```python
from build123d import *

# Parameters (mm, degrees)
SKETCH1_W           = 100
SKETCH1_H           = 40
BOSS_EXTRUDE1_DEPTH = 10
SKETCH2_R           = 12
CUT_EXTRUDE1_DEPTH  = 10
FILLET1_R           = 10
CUT_EXTRUDE2_DEPTH  = 10
BOSS_EXTRUDE2_START = 60
SKETCH4_R           = 20
BOSS_EXTRUDE2_DEPTH = 60
SKETCH5_R           = 40
BOSS_EXTRUDE3_DEPTH = 20


with BuildPart() as part:
    # Sketch1 → Boss-Extrude1 (new body)
    with BuildSketch(Plane.XY):
        Rectangle(SKETCH1_W, SKETCH1_H)
    extrude(amount=BOSS_EXTRUDE1_DEPTH)

    # Sketch2 → Cut-Extrude1 (cut)
    with BuildSketch(Plane.XY.offset(10)):
        with Locations((30, 0)):
            Circle(SKETCH2_R)
    extrude(amount=-CUT_EXTRUDE1_DEPTH, mode=Mode.SUBTRACT)

    # Fillet1
    fillet1_edges = [part.edges().sort_by_distance(p)[0] for p in [
        (50, -20, 5),
        (50, 20, 5),
    ]]
    fillet(fillet1_edges, radius=FILLET1_R)

    # Sketch3 → Cut-Extrude2 (cut)
    with BuildSketch(Plane(origin=(0, 0, 0), x_dir=(-1, 0, 0), z_dir=(0, 0, -1))):
        with BuildLine():
            Line((50, 20), (30, 20))
            ThreePointArc((30, 20), (44.142135624, 14.142135624), (50, 0))
            Line((50, 0), (50, 20))
        make_face()
        with BuildLine():
            Line((50, -20), (50, 0))
            ThreePointArc((50, 0), (44.142135624, -14.142135624), (30, -20))
            Line((30, -20), (50, -20))
        make_face()
    extrude(amount=-CUT_EXTRUDE2_DEPTH, mode=Mode.SUBTRACT)

    # Sketch4 → Boss-Extrude2 (add)
    with BuildSketch(Plane(origin=(0, 0, 0), x_dir=(-1, 0, 0), z_dir=(0, 0, -1)).offset(BOSS_EXTRUDE2_START)):
        with Locations((30, 0)):
            Circle(SKETCH4_R)
    extrude(amount=-BOSS_EXTRUDE2_DEPTH)

    # Sketch5 → Boss-Extrude3 (add)
    with BuildSketch(Plane(origin=(0, 0, 0), x_dir=(-1, 0, 0), z_dir=(0, 0, -1))):
        with Locations(Location((30, 0, 0), (0, 0, 210))):
            Circle(SKETCH5_R)
    extrude(amount=BOSS_EXTRUDE3_DEPTH)


solid = part.part
```
Can you work these out from the model? Positions are in its coordinate system, mm. A direction names the side the tool comes from. Give positions to 0.01 mm unless a question says otherwise; leave off trailing zeros. Loops run counter-clockwise (first coordinate to the right, second up) from the corner with the lowest first, then second, coordinate; pieces in that order, holes last. Notation, with made-up numbers: M 42.25,77 L 99.25,77 A29 ccw 99.25,99 Z; hole C 19.25,57 d5. An arc over 180 degrees is marked long. Use one line per item in the form item = value. Start each with the question number.
(1) I want a section at C-C, the plane y = 17.5. Write out the boundary of the cut face in (x, z), and give its area (3 significant figures).
(2) Thinking about a two-plate mould opening in Y: for faces 6 (the cylindrical face through (46.99, 17.15, 5.07)), 7 (the cylindrical face through (41.085, -4.596, 5.07)), 8 (the cylindrical face through (46.99, -17.15, 5.07)), 9 (the flat face through (-51, 1, 0)), which applies, released by +Y, released by -Y, zero draft, split by the parting line, or undercut?
(3) On a 3-axis mill with a long thin cutter (end or side, diameter ignored), from which of +Z, -Z, +X, -X, +Y, -Y can I reach the whole of each face in a straight line? I mean faces 1 (the flat face through (5, -20, 5)), 2 (the flat face through (-30, 0, -60)), 3 (the cylindrical face through (-49.076, 6.007, -40.28)), 4 (the flat face through (5, 20, 5)), 5 (the flat face through (50, 0, 5)). Say none if no direction works.
(4) Please list where these lines run through material, in increasing order: line 1 (Y direction, x = 30.5, z = 7); line 2 (Z direction, x = -7.5, y = -26); line 3 (X direction, y = 5, z = 5).
(5) I want a section at D-D, the plane x = -42.5. Write out the boundary of the cut face in (y, z).
(6) I want a section at A-A, the plane x = 30. Write out the boundary of the cut face in (y, z), and give its area (3 significant figures).
(7) I want a section at B-B, the plane z = -17. Write out the boundary of the cut face in (x, y), and give its area (3 significant figures).
(8) I'm going to push flat-ended pins straight in: P1, Ø12, axis at x = -45, y = 15.5, coming from the +Z side; P2, Ø10, axis at x = -48, y = -24, coming from the +Z side; P3, Ø1, axis at y = -28, z = 1.5, coming from the +X side (3 decimals); P4, Ø10, axis at x = -53.5, y = 23, coming from the -Z side. Where does each tip first touch, or does it pass through?
Worked out:
q1.outline = M -65.97,-20 L -39.68,-20 L -39.68,-60 L -20.32,-60 L -20.32,-20 L 5.97,-20 L 5.97,0 L 46.61,0 L 46.61,10 L -39.68,10 L -39.68,0 L -65.97,0 Z
q1.area = 3,080 mm²
q2.face_6 = released by +Y
q2.face_7 = undercut
q2.face_8 = released by -Y
q2.face_9 = zero draft
q3.face_1 = +Z, +X, -X, -Y
q3.face_2 = -Z, +X, -X, +Y, -Y
q3.face_3 = -Z
q3.face_4 = +Z, +X, -X, +Y
q3.face_5 = +Z, -Z, +X, +Y, -Y
q4.line_1 = -20 to -11.99, 11.99 to 20
q4.line_2 = -20 to 0
q4.line_3 = -49.36 to 19.09, 40.91 to 50
q5.outline = M -38,-20 L -15.61,-20 L -15.61,-60 L 15.61,-60 L 15.61,-20 L 38,-20 L 38,0 L 15.61,0 L 15.61,10 L -15.61,10 L -15.61,0 L -38,0 Z
q6.outline = M -20,0 L -12,0 L -12,10 L -20,10 Z; M 12,0 L 20,0 L 20,10 L 12,10 Z
q6.area = 160 mm²
q7.outline = C -30,0 d80
q7.area = 5,030 mm²
q8.P1 = 10
q8.P2 = 0
q8.P3 = through
q8.P4 = -20
